Model file for the job. Use its own axes, mm. A direction names the side the tool comes from. Round coordinates to 2 decimals unless told otherwise and drop trailing zeros.
from build123d import *

# Parameters (mm, degrees)
SKETCH2_R           = 120
CUT_EXTRUDE1_DEPTH  = 5
CUT_EXTRUDE2_START  = -5
SKETCH3_R           = 120
CUT_EXTRUDE2_DEPTH  = 5
SKETCH4_R           = 8
CUT_EXTRUDE3_DEPTH  = 202.944299251
BOSS_EXTRUDE1_START = 5
SKETCH5_R           = 22.870444207
SKETCH5_R_2         = 8
BOSS_EXTRUDE1_DEPTH = 5
SKETCH6_R           = 22.870444207
SKETCH6_R_2         = 8
BOSS_EXTRUDE2_DEPTH = 5
CUT_EXTRUDE5_DEPTH  = 202.944299251
CIRPATTERN1_COUNT   = 4


with BuildPart() as part:
    # Sketch1 → Revolve1 (revolve)
    with BuildSketch(Plane(origin=(0, 0, 0), x_dir=(1, 0, 0), z_dir=(0, 1, 0)), mode=Mode.PRIVATE) as revolve1_sk:
        Polygon((0, 0), (0, 142.5), (1.439897502, 142.5), (3.207174134, 138.107099477), (5.784452556, 138.107099477), (7.10991003, 142.5), (11.012645925, 142.5), (12.264466873, 138.107099477), (14.915381821, 138.107099477), (16.240839295, 142.5), (18, 142.5), (18, 0), align=None)
    revolve(revolve1_sk.sketch.rotate(Axis((0, 0, 0), (1, 0, 0)), 180), axis=Axis((0, 0, 0), (1, 0, 0)))

    # Sketch2 → Cut-Extrude1 (cut)
    with BuildSketch(Plane.ZY):
        Circle(SKETCH2_R)
    extrude(amount=-CUT_EXTRUDE1_DEPTH, mode=Mode.SUBTRACT)

    # Sketch3 → Cut-Extrude2 (cut)
    with BuildSketch(Plane(origin=(18, 0, 0), x_dir=(0, 0, -1), z_dir=(1, 0, 0)).offset(CUT_EXTRUDE2_START)):
        with Locations(Location((0, 0, 0), (0, 0, 180))):
            Circle(SKETCH3_R)
    extrude(amount=CUT_EXTRUDE2_DEPTH, mode=Mode.SUBTRACT)

    # Sketch4 → Cut-Extrude3 (cut, through all)
    with BuildSketch(Plane(origin=(13, 0, 0), x_dir=(0, 0, -1), z_dir=(1, 0, 0))):
        Circle(SKETCH4_R)
    extrude(amount=-CUT_EXTRUDE3_DEPTH, mode=Mode.SUBTRACT)

    # Sketch5 → Boss-Extrude1 (add)
    with BuildSketch(Plane(origin=(13, 0, 0), x_dir=(0, 0, -1), z_dir=(1, 0, 0)).offset(BOSS_EXTRUDE1_START)):
        Circle(SKETCH5_R)
        Circle(SKETCH5_R_2, mode=Mode.SUBTRACT)
    extrude(amount=-BOSS_EXTRUDE1_DEPTH)

    # Sketch6 → Boss-Extrude2 (add)
    with BuildSketch(Plane.ZY.offset(-5)):
        with Locations(Location((0, 0, 0), (0, 0, 180))):
            Circle(SKETCH6_R)
        with Locations(Location((0, 0, 0), (0, 0, 180))):
            Circle(SKETCH6_R_2, mode=Mode.SUBTRACT)
    extrude(amount=BOSS_EXTRUDE2_DEPTH)

    # Sketch7 → Cut-Extrude5 (cut, through all)
    with BuildSketch(Plane.ZY.offset(-5)):
        with BuildLine():
            Line((-5.40203869, 35.175568579), (-5.40203869, 110.423122323))
            ThreePointArc((-5.40203869, 110.423122323), (-77.592767083, 78.751574346), (-110.330916303, 7.038243628))
            Line((-110.330916303, 7.038243628), (-34.885036528, 7.038243628))
            ThreePointArc((-34.885036528, 7.038243628), (-24.57009099, 25.745160237), (-5.40203869, 35.175568579))
        make_face()
    cut_extrude5 = extrude(amount=-CUT_EXTRUDE5_DEPTH, mode=Mode.SUBTRACT)

    # CirPattern1: Cut-Extrude5 ×4 about axis
    cirpattern1_axis = Axis((0, 0, 0), (1, 0, 0))
    for i in range(1, CIRPATTERN1_COUNT):
        add(cut_extrude5.rotate(cirpattern1_axis, i * 360 / CIRPATTERN1_COUNT), mode=Mode.SUBTRACT)


solid = part.part
Q1. Flat gauge pins, fed straight in: P1, Ø9, axis at x = 8, z = -55.5, coming from the +Y side; P2, Ø6.5, axis at x = 8, y = 75, coming from the -Z side; P3, Ø4, axis at x = 7.5, z = -73.5, coming from the -Y side; P4, Ø4, axis at y = -92.5, z = 54.5, coming from the -X side. Where does each tip first touch, or does it go through?
Q2. Probe line 1 (Y direction, x = 14.55, z = 0); line 2 (Z direction, x = 8, y = -53.5); line 3 (Y direction, x = 16.65, z = 0). List the from-to ranges inside material, lowest first.
Q3. Pull direction Y, two halves, no side cores. Call faces 5 (the face through (0, 94, 75)), 6 (the face through (9, -72, 5.402)), 7 (the face through (0.73, -96.308, -105.028)): pulls with the +Y half, pulls with the -Y half, needs draft (parallel to the pull), parting line crosses it, or undercut.
Q4. Tool access for faces 1 (the face through (2.465, 5.276, -119.884)), 2 (the face through (8.944, -79.539, 76.785)), 3 (the face through (18, 94, -75)), 4 (the face through (5.867, -41.566, 131.992)): list every direction of +Z, -Z, +X, -X, +Y, -Y with a clear straight run to the whole face (end or side of a thin tool).
Q5. Slice it at A-A on z = -83.5. State how many separate pieces and enclosed holes the cut face has, plus the area to 3 significant figures.
Reply:
1. P1: stops at y = 133.06
1. P2: stops at z = -123.12
1. P3: stops at y = -123.26
1. P4: passes through
2. line 1: y = -138.11 to -120, -22.87 to -8, 8 to 22.87, 120 to 138.11
2. line 2: z = -132.08 to -96.75, -7.04 to 5.4, 96.75 to 132.08
2. line 3: y = -142.5 to -120, -22.87 to -8, 8 to 22.87, 120 to 142.5
3. face 5: needs draft
3. face 6: undercut
3. face 7: parting line crosses it
4. face 1: -X
4. face 2: +X, -X
4. face 3: +Z, -Z, +X, +Y, -Y
4. face 4: none
5. separate pieces: 3
5. enclosed holes: 0
5. area: 1,290 mm2
